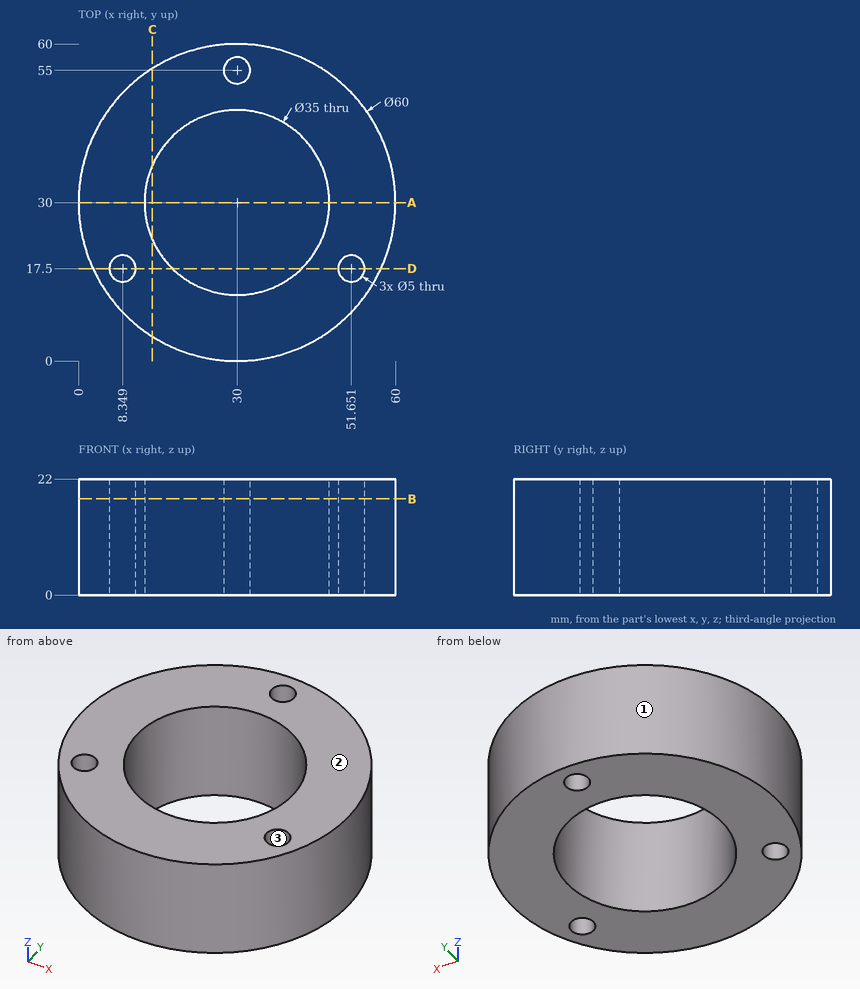
Drawing for the job (mm, zero at the part's lowest x, y, z). Round coordinates to 2 decimals unless told otherwise and drop trailing zeros. Order: outer loops, then holes, each group sorted by start corner. A loop starts at its lowest first (then second) coordinate and runs counter-clockwise, first axis right, second up.
Item 1: Saw through at B-B on z = 18.25. Write the cut outline in (x, y), then the cut area to 3 significant figures.
Item 2: Pin check, flat tips, straight feed: pin 1 (3 mm diameter, centred on y = 47, z = 4, fed in from +X) (1 decimal); pin 2 (1 mm diameter, centred on x = 25, z = 7, fed in from -Y); pin 3 (12 mm diameter, centred on x = 29, z = 13.5, fed in from -Y); pin 4 (8 mm diameter, centred on x = 51.65, y = 17.5, fed in from -Z). Stop position of each tip, or through.
Item 3: Saw through at A-A on y = 30. Write the cut outline in (x, z).
Item 4: Saw through at D-D on y = 17.5. Write the cut outline in (x, z), then the cut area to 3 significant figures.
Item 5: Saw through at C-C on x = 14. Write the cut outline in (y, z), then the cut area to 3 significant figures.
Item 6: Probe line 1 along Y through (x, z) = (30, 12.5); line 2 along X through (y, z) = (18.5, 6.75); line 3 along X through (y, z) = (16.5, 14) (1 decimal). List the from-to ranges inside material, lowest first.
Item 7: Mould opens along X. For the marked faces 1, 2 and 3 say: pulls with the +X half, pulls with the -X half, needs draft (parallel to the pull), parting line crosses it, or undercut.
Reported:
1. outline: circle Ø60 at (30, 30); hole circle Ø5 at (8.35, 17.5); hole circle Ø35 at (30, 30); hole circle Ø5 at (30, 55); hole circle Ø5 at (51.65, 17.5)
1. area: 1,810 mm2
2. pin 1: stops at x = 55.7
2. pin 2: stops at y = 0.34
2. pin 3: stops at y = 0
2. pin 4: stops at z = 0
3. outline: (0, 0) - (12.5, 0) - (12.5, 22) - (0, 22) - close; (47.5, 0) - (60, 0) - (60, 22) - (47.5, 22) - close
4. outline: (2.73, 0) - (5.85, 0) - (5.85, 22) - (2.73, 22) - close; (10.85, 0) - (17.75, 0) - (17.75, 22) - (10.85, 22) - close; (42.25, 0) - (49.15, 0) - (49.15, 22) - (42.25, 22) - close; (54.15, 0) - (57.27, 0) - (57.27, 22) - (54.15, 22) - close
4. area: 441 mm2
5. outline: (4.62, 0) - (22.91, 0) - (22.91, 22) - (4.62, 22) - close; (37.09, 0) - (55.38, 0) - (55.38, 22) - (37.09, 22) - close
5. area: 805 mm2
6. line 1: y = 0 to 12.5, 47.5 to 52.5, 57.5 to 60
6. line 2: x = 2.29 to 6.06, 10.64 to 16.81, 43.19 to 49.36, 53.94 to 57.71
6. line 3: x = 3.2 to 6.1, 10.6 to 18.9, 41.1 to 49.4, 53.9 to 56.8
7. face 1: parting line crosses it
7. face 2: needs draft
7. face 3: undercut
